Geometry: see drawing. Coordinates: mm, zero at the bounding-box minimum. A direction names the side the tool comes from. Coordinates: 2 decimals unless noted, no trailing zeros. Write each loop counter-clockwise with the first axis right and the second up, starting at its lowest first coordinate (ties: lowest second). Pieces come first, ordered by that corner, then holes. Notation, with made-up numbers: (-11.5, -29) - (-3.5, -29) arc R14 cw to (-3.5, -20) - close; hole circle Ø6 at (-15, 55.25). An arc over 180 degrees is marked (long way). One line per question, with ' | ' between items. Start each with the question number.
Q1. Contact query for flat-ended pins moving along their axis: P1, Ø1.5, axis at y = 11, z = 15.5, coming from the -X side; P2, Ø10, axis at x = 53.5, y = 23.5, coming from the +Z side; P3, Ø6.5, axis at x = 8, y = 12.5, coming from the +Z side; P4, Ø3, axis at x = 52, z = 60, coming from the +Y side. Output: stop coordinate, or through.
Q2. Cut plane B-B, the plane y = 14. Return loops of the section in (x, z).
Q3. Draft query along X for the marked faces 6, 7, 8 and 9. Return one class per face: +X half, -X half, draft (parallel to the pull), parting line (faces both ways), or undercut.
Q4. Cut plane A-A, the plane x = 36. Return loops of the section in (y, z), plus the area to 3 significant figures.
Q5. Access query for the marked faces 1, 2, 3, 4 and 5. Directions: +Z, -Z, +X, -X, +Y, -Y. A direction counts if a zero-diameter tool reaches every point of the face in a straight line with its end or side. Return the directions, or none.
Q6. Line query: line 1 (Y direction, x = 60, z = 4.5); line 2 (Z direction, x = 49.5, y = 4); line 3 (X direction, y = 7.5, z = 8) (1 decimal). Output: solid intervals per line, ascending.
Q7. Cut plane D-D, the plane x = 24. Return loops of the section in (y, z), plus the area to 3 significant figures.
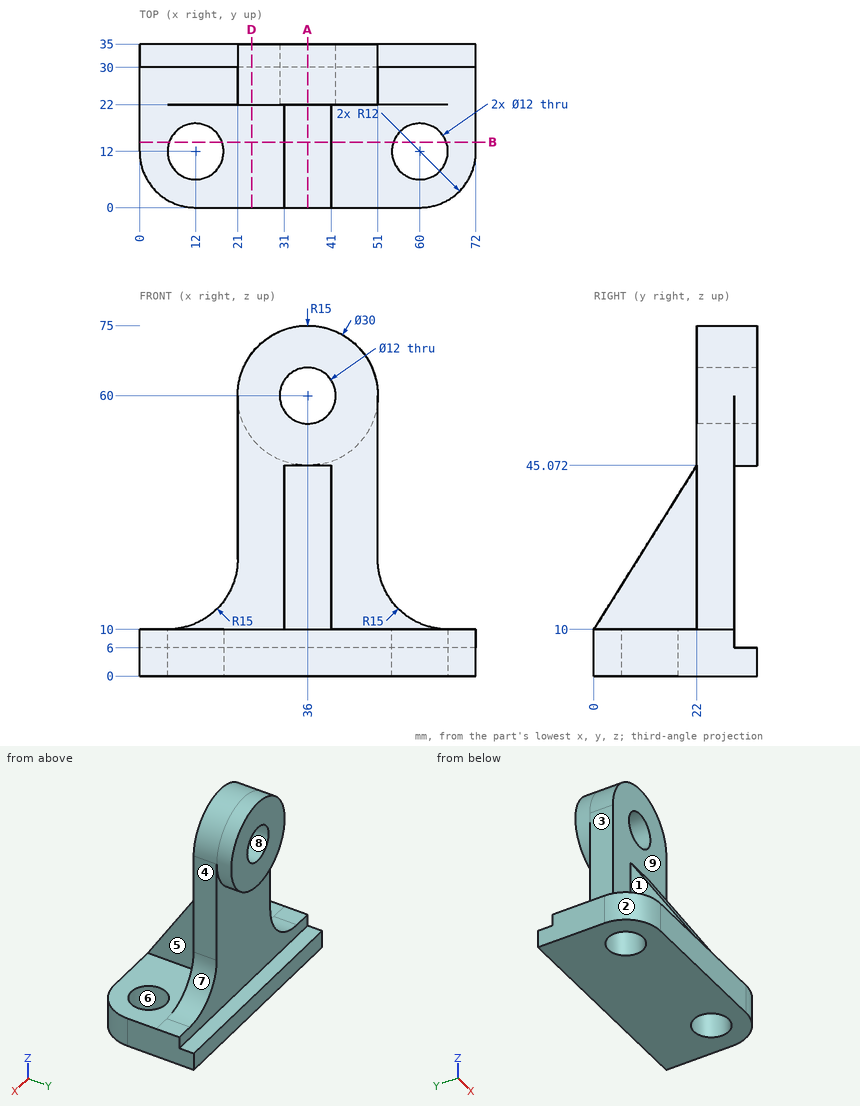
Reply:
1) P1: stops at x = 31 | P2: stops at z = 68.29 | P3: stops at z = 10 | P4: stops at y = 35
2) outline: (0, 0) - (6.34, 0) - (6.34, 10) - (0, 10) - close; (17.66, 0) - (54.34, 0) - (54.34, 10) - (41, 10) - (41, 32.32) - (31, 32.32) - (31, 10) - (17.66, 10) - close; (65.66, 0) - (72, 0) - (72, 10) - (65.66, 10) - close
3) face 6: undercut | face 7: +X half | face 8: undercut | face 9: draft
4) outline: (0, 0) - (35, 0) - (35, 6) - (30, 6) - (30, 45) - (35, 45) - (35, 54) - (22, 54) - (22, 45.07) - (0, 10) - close; (22, 66) - (35, 66) - (35, 75) - (22, 75) - close | area: 1,230 mm^2
5) face 1: +Z, -X, -Y | face 2: +Z, -Z, -X, -Y | face 3: +Z, -X, +Y, -Y | face 4: +Z, +X, +Y, -Y | face 5: +Z, +X, -Y
6) line 1: y = 0 to 6, 18 to 35 | line 2: z = 0 to 10 | line 3: x = 0.9 to 8, 16 to 56, 64 to 71.1
7) outline: (0, 0) - (35, 0) - (35, 6) - (30, 6) - (30, 51) - (35, 51) - (35, 69) - (22, 69) - (22, 10) - (0, 10) - close | area: 892 mm^2
